from build123d import *

# Parameters (mm, degrees)
SKETCH1_R         = 5.188
BASENUT_DEPTH     = 12
EXTRUDE1_START    = 0.6
SKETCH3_R         = 8.315
SKETCH3_R_2       = 5.188
EXTRUDE1_DEPTH    = 0.6
ENDCHAMFER3_SIZE  = 1.312
ENDCHAMFER3_SIZE2 = 0.757483553


with BuildPart() as part:
    # Sketch1 → BaseNut (new body)
    with BuildSketch(Plane.XY):
        Polygon((5.196152423, -9), (10.392304845, 0), (5.196152423, 9), (-5.196152423, 9), (-10.392304845, 0), (-5.196152423, -9), align=None)
        Circle(SKETCH1_R, mode=Mode.SUBTRACT)
    extrude(amount=-BASENUT_DEPTH)

    # Sketch2 → Chamfer1 (revolve, cut)
    with BuildSketch(Plane(origin=(-16.706149795, 0, -15.04811501), x_dir=(0, 0, 1), z_dir=(0, 1, 0))):
        Polygon((3.04811501, 25.706149795), (3.04811501, 27.098454641), (3.851962587, 27.098454641), align=None)
    revolve(axis=Axis((0, 0, -38.770766557), (0, 0, 1)), mode=Mode.SUBTRACT)

    # Sketch6 → EndChamfer1 (revolve, cut)
    with BuildSketch(Plane(origin=(-9.197458863, 0, -10.252541137), x_dir=(0, 0, 1), z_dir=(0, 1, 0))):
        Polygon((-1.747458863, 14.385458863), (-1.747458863, 15.697458863), (-0.989975309, 14.385458863), align=None)
    revolve(axis=Axis((0, 0, 13.104863586), (0, 0, -1)), mode=Mode.SUBTRACT)

    # Sketch3 → Extrude1 (add)
    with BuildSketch(Plane(origin=(-18.48918612, 11.17895969, 0), x_dir=(1, 0, 0), z_dir=(0, 0, 1)).offset(EXTRUDE1_START)):
        with Locations((18.48918612, -11.17895969)):
            Circle(SKETCH3_R)
        with Locations((18.48918612, -11.17895969)):
            Circle(SKETCH3_R_2, mode=Mode.SUBTRACT)
    extrude(amount=-EXTRUDE1_DEPTH)

    # EndChamfer3
    endchamfer3_edges = [part.edges().sort_by_distance(p)[0] for p in [
        (-5.188, 0, 0.6),
    ]]
    endchamfer3_side = [part.faces().sort_by_distance(p)[0] for p in [
        (-8.079816285, 0, 0.6),
    ]]
    chamfer(endchamfer3_edges, length=ENDCHAMFER3_SIZE, length2=ENDCHAMFER3_SIZE2, reference=endchamfer3_side[0])


solid = part.part
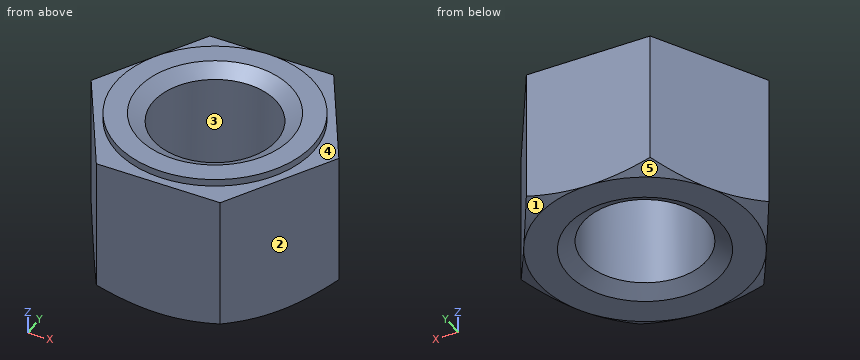
Read the model definition and answer for the solid it produces. Units are mm, in the model's axes. Face numbers are marked on the shaded views. A direction names the side the tool comes from. Give positions to 0.01 mm unless a question says otherwise; leave off trailing zeros. Loops run counter-clockwise (first coordinate to the right, second up) from the corner with the lowest first, then second, coordinate; pieces in that order, holes last. Notation, with made-up numbers: M -1.75,79 L 48.25,79 A10 cw 48.25,90 Z; hole C 64.25,5 d6. An arc over 180 degrees is marked long. Write each question's results on one line, items separated by ' | '.
1. Straight lines are drawn through the part: line 1 (Y direction, x = 0, z = -5.25); line 2 (X direction, y = 1.75, z = -9.75); line 3 (X direction, y = 4.25, z = -0.25). For each, find the intervals that lie inside material, in ascending order. Write a range as [from, to].
Values:
line 1: y = [-9, -5.19], [5.19, 9] | line 2: x = [-9.38, -4.88], [4.88, 9.38] | line 3: x = [-7.94, -2.98], [2.98, 7.94]
2. Given pin 1 (3 mm diameter, centred on y = -4.5, z = -6, fed in from -X); pin 2 (6 mm diameter, centred on y = -1, z = -8.5, fed in from -X); pin 3 (3 mm diameter, centred on y = 3.5, z = -1.5, fed in from -X); pin 4 (3 mm diameter, centred on x = 4, y = -2, fed in from -Z), each flat-ended and moving along its own axis, determine where each tip first touches the part or whether it passes through.
Values:
pin 1: stops at x = -8.66 | pin 2: stops at x = -10.39 | pin 3: stops at x = -9.24 | pin 4: stops at z = -11.7
3. Section A-A on z = -7.25 is taken. Give the vertices of the cut face in (x, y), plus the area to 3 significant figures.
Values:
outline: M -10.39,0 L -5.2,-9 L 5.2,-9 L 10.39,0 L 5.2,9 L -5.2,9 Z; hole C 0,0 d10.38 | area: 196 mm^2
4. A tool of negligible diameter and unlimited length cuts with its end or side. For the marked faces 4 and 5, from which of +Z, -Z, +X, -X, +Y, -Y can it reach the whole face along a straight path? Write none if from no direction.
Values:
face 4: +Z | face 5: -Z, -X, +Y
5. The mould has two halves that part along Y. Classify the marked faces 1, 2 and 3: pulls with the +Y half, pulls with the -Y half, needs draft (parallel to the pull), parting line crosses it, or undercut.
Values:
face 1: pulls with the +Y half | face 2: pulls with the -Y half | face 3: undercut
